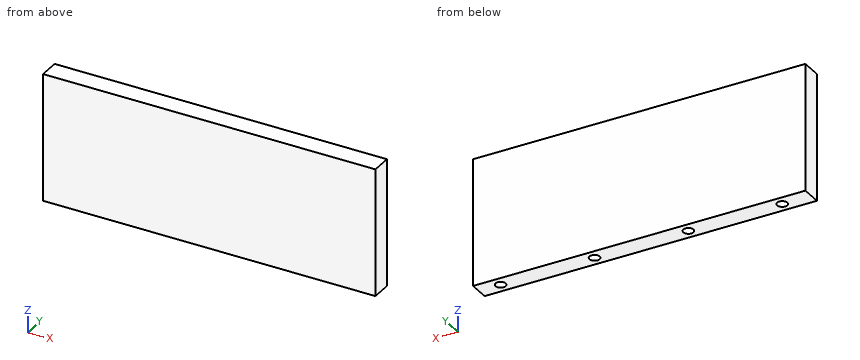
```python
from build123d import *

# Parameters (mm, degrees)
SKETCH1_W           = 131
SKETCH1_H           = 8
BOSS_EXTRUDE1_DEPTH = 50
SKETCH2_R           = 2
CUT_EXTRUDE1_DEPTH  = 15


with BuildPart() as part:
    # Sketch1 → Boss-Extrude1 (new body)
    with BuildSketch(Plane.XY):
        with Locations((65.5, 4)):
            Rectangle(SKETCH1_W, SKETCH1_H)
    extrude(amount=BOSS_EXTRUDE1_DEPTH)

    # Sketch2 → Cut-Extrude1 (cut)
    with BuildSketch(Plane(origin=(0, 0, 0), x_dir=(-1, 0, 0), z_dir=(0, 0, -1))):
        with Locations((-122.391171487, 4)):
            Circle(SKETCH2_R)
        with Locations((-85.391171487, 4)):
            Circle(SKETCH2_R)
        with Locations((-48.391171487, 4)):
            Circle(SKETCH2_R)
        with Locations((-11.391171487, 4)):
            Circle(SKETCH2_R)
    extrude(amount=-CUT_EXTRUDE1_DEPTH, mode=Mode.SUBTRACT)


solid = part.part
```
CAD build for the part. Positions are in the model's coordinates, mm. Round coordinates to 2 decimals unless told otherwise and drop trailing zeros. Loops run counter-clockwise (first coordinate to the right, second up) from the corner with the lowest first, then second, coordinate; pieces in that order, holes last. Notation, with made-up numbers: M 28.5,-30 L 69.5,-30 A7 ccw 69.5,-17 Z; hole C 54,0.5 d11. An arc over 180 degrees is marked long. Return JSON: item names as keys, results as strings. Group by question number.
(1) Wall check: probe 1 along X at (y, z) = (2.5, 9.5); probe 2 along X at (y, z) = (5.75, 10); probe 3 along Z at (x, y) = (50, 3.75). Give the ranges that are in metal, low to high. Write a range as [from, to].
(2) Drop a flat-ended pin along its axis: P1, Ø1.2, axis at x = 122, y = 3.5, coming from the -Z side. Give the stop position or say it passes through.
(3) Saw through at C-C, the plane x = 123. List the corners of the cut face in (y, z).
(4) Saw through at B-B, the plane y = 4. List the corners of the cut face in (x, z), and give its area (3 significant figures).
(5) Saw through at A-A, the plane z = 7. List the corners of the cut face in (x, y).
Answer list:
{
 "1": {"probe 1": "[0, 10.07], [12.71, 47.07], [49.71, 84.07], [86.71, 121.07], [123.71, 131]", "probe 2": "[0, 10.42], [12.36, 47.42], [49.36, 84.42], [86.36, 121.42], [123.36, 131]", "probe 3": "[15, 50]"},
 "2": {"P1": "z = 15"},
 "3": {"outline": "M 0,0 L 2.09,0 L 2.09,15 L 5.91,15 L 5.91,0 L 8,0 L 8,50 L 0,50 Z"},
 "4": {"outline": "M 0,0 L 9.39,0 L 9.39,15 L 13.39,15 L 13.39,0 L 46.39,0 L 46.39,15 L 50.39,15 L 50.39,0 L 83.39,0 L 83.39,15 L 87.39,15 L 87.39,0 L 120.39,0 L 120.39,15 L 124.39,15 L 124.39,0 L 131,0 L 131,50 L 0,50 Z", "area": "6,310 mm2"},
 "5": {"outline": "M 0,0 L 131,0 L 131,8 L 0,8 Z; hole C 11.39,4 d4; hole C 48.39,4 d4; hole C 85.39,4 d4; hole C 122.39,4 d4"}
}
